Design review of the part built by this model. Coordinates are the model's own, in mm. A direction names the side the tool comes from. Give positions to 0.01 mm unless a question says otherwise; leave off trailing zeros. Order: outer loops, then holes, each group sorted by start corner. A loop starts at its lowest first (then second) coordinate and runs counter-clockwise, first axis right, second up. Notation, with made-up numbers: M 7,34.25 L 13,34.25 A34 cw 13,72.25 Z; hole C -32,-37 d3. An arc over 180 degrees is marked long. Put each result on its own line as item: value. Start each with the question number.
from build123d import *

# Parameters (mm, degrees)
BOSS_EXTRUDE1_DEPTH = 6.4
SKETCH4_R           = 17.59
SKETCH4_R_2         = 8
CUT_EXTRUDE1_DEPTH  = 0.8
CUT_EXTRUDE1_DRAFT  = -60
CHAMFER2_SIZE       = 0.555555556


with BuildPart() as part:
    # Sketch3 → Boss-Extrude1 (new body)
    with BuildSketch(Plane(origin=(0, 0, 0), x_dir=(0, 0, -1), z_dir=(1, 0, 0))):
        Polygon((8, 4.618802154), (0, 9.237604307), (-8, 4.618802154), (-8, -4.618802154), (0, -9.237604307), (8, -4.618802154), align=None)
    extrude(amount=BOSS_EXTRUDE1_DEPTH)


with BuildPart() as cut_extrude1_tool:
    # Sketch4 → Cut-Extrude1 (with draft: the straight prism first)
    with BuildSketch(Plane.ZY):
        Circle(SKETCH4_R)
        Circle(SKETCH4_R_2, mode=Mode.SUBTRACT)
    extrude(amount=-CUT_EXTRUDE1_DEPTH)
    # Cut-Extrude1: the draft: its side faces are tilted about the plane it starts from
    cut_extrude1_sides = [cut_extrude1_tool.faces().sort_by_distance(p)[0] for p in [
        (0.4, 0, -17.59),
        (0.4, 0, -8),
    ]]
    draft(cut_extrude1_sides, Plane.ZY, CUT_EXTRUDE1_DRAFT)


with BuildPart() as part_1:
    add(part.part)

    # Cut-Extrude1: cut by cut_extrude1_tool
    add(cut_extrude1_tool.part, mode=Mode.SUBTRACT)

    # Sketch5 → Revolve1 (revolve)
    with BuildSketch(Plane.XY, mode=Mode.PRIVATE) as revolve1_sk:
        with BuildLine():
            Line((7.5, 5), (36.4, 5))
            Line((36.4, 5), (36.4, 0))
            Line((36.4, 0), (6.4, 0))
            Line((6.4, 0), (6.4, 6.1))
            ThreePointArc((6.4, 6.1), (6.722182541, 5.322182541), (7.5, 5))
        make_face()
    revolve(revolve1_sk.sketch.rotate(Axis((6.4, 0, 0), (1, 0, 0)), 90), axis=Axis((6.4, 0, 0), (1, 0, 0)))

    # Chamfer2
    chamfer2_edges = [part_1.edges().sort_by_distance(p)[0] for p in [
        (36.4, 0, -5),
    ]]
    chamfer(chamfer2_edges, length=CHAMFER2_SIZE)


solid = part_1.part
1. Insertion check: pin 1 (2 mm diameter, centred on y = -4.5, z = 4, fed in from -X); pin 2 (8 mm diameter, centred on x = 19.5, z = 2, fed in from +Y); pin 3 (4 mm diameter, centred on x = 12.5, y = -2, fed in from -Z); pin 4 (2 mm diameter, centred on x = 22.5, y = 4.5, fed in from -Z). Each pin has a flat end and moves straight along its axis. Give the tip position at first contact, or say it passes through.
2. Machinability: for faces 1 (the cylindrical face through (22, 0, -5)), 2 (the conical face through (0.17, 4.13, 7.19)), which of the approach directions +Z, -Z, +X, -X, +Y, -Y give a long, thin tool a straight path to every point of the face, cutting with its end or side? Answer none if there is none.
3. Consider section A-A on x = 2.5. Give the boundary of the cut face in (y, z).
4. To check wall thickness, follow probe 1 along X at (y, z) = (-6, -2.25); probe 2 along Z at (x, y) = (29, 3); probe 3 along X at (y, z) = (4, 3.5). State the ranges of each line that lie inside material, in increasing order.
5. Consider section B-B on x = 9. Give the boundary of the cut face in (y, z), then the cut area to 3 significant figures.
Returned:
1. pin 1: stops at x = 0
1. pin 2: stops at y = 5
1. pin 3: stops at z = -5
1. pin 4: stops at z = -3.57
2. face 1: +X
2. face 2: +Z, -X, +Y
3. outline: M -9.24,0 L -4.62,-8 L 4.62,-8 L 9.24,0 L 4.62,8 L -4.62,8 Z
4. probe 1: x = 0 to 6.4
4. probe 2: z = -4 to 4
4. probe 3: x = 0 to 6.73
5. outline: C 0,0 d10
5. area: 78.5 mm2
